The figure shows three views and two pictorial views of one solid part (mm, origin at its lowest corner). Answer the questions. Coordinates: 2 decimals unless noted, no trailing zeros. Order: outer loops, then holes, each group sorted by start corner. A loop starts at its lowest first (then second) coordinate and runs counter-clockwise, first axis right, second up. Notation, with made-up numbers: M 81,6 L 131,6 A10 cw 131,10 Z; hole C 68.5,2 d10. An arc over 180 degrees is marked long. Use a Markdown table: item, result.
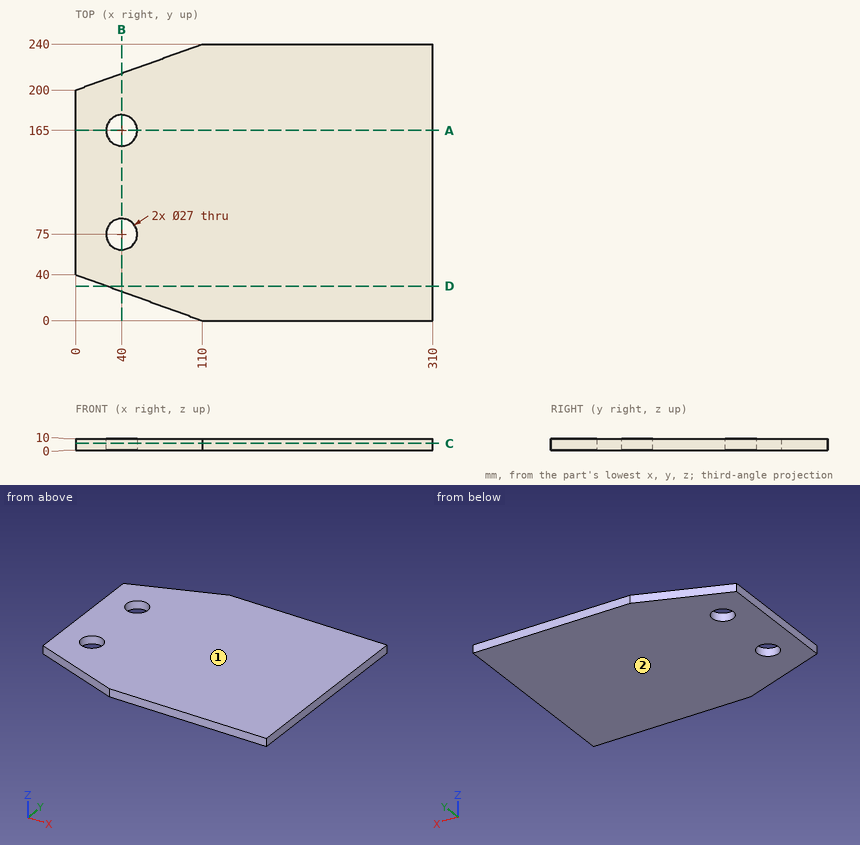
1. For a pull along Z with two mould halves and no side action, classify the marked faces 1 and 2 as +Z half, -Z half, draft (parallel to the pull), parting line (faces both ways), or undercut.
Answers below:
| item | result |
|---|---|
| face 1 | +Z half |
| face 2 | -Z half |
2. Section A-A on y = 165 is taken. Determine the outline of the cut face in (x, z), then the cut area to 3 significant figures.
Answers below:
| item | result |
|---|---|
| outline | M 0,0 L 26.5,0 L 26.5,10 L 0,10 Z; M 53.5,0 L 310,0 L 310,10 L 53.5,10 Z |
| area | 2,830 mm² |
3. Find the intervals of material crossed by probe 1 along Y at (x, z) = (40, 5.5); probe 2 along X at (y, z) = (164.5, 4.5); probe 3 along X at (y, z) = (73.5, 1.5), in increasing order.
Answers below:
| item | result |
|---|---|
| probe 1 | 25.45 to 61.5, 88.5 to 151.5, 178.5 to 214.55 |
| probe 2 | 0 to 26.51, 53.49 to 310 |
| probe 3 | 0 to 26.58, 53.42 to 310 |
4. Section C-C on z = 6 is taken. Determine the outline of the cut face in (x, y).
Answers below:
| item | result |
|---|---|
| outline | M 0,40 L 110,0 L 310,0 L 310,240 L 110,240 L 0,200 Z; hole C 40,75 d27; hole C 40,165 d27 |
5. A flat-ended cylindrical pin translates along its axis: P1, Ø21.5, axis at x = 40, y = 165, coming from the +Z side. Find the tip coordinate at first contact, or state that the pin passes through.
Answers below:
| item | result |
|---|---|
| P1 | through |
6. Section D-D on y = 30 is taken. Determine the outline of the cut face in (x, z).
Answers below:
| item | result |
|---|---|
| outline | M 27.5,0 L 310,0 L 310,10 L 27.5,10 Z |
7. Section B-B on x = 40 is taken. Determine the outline of the cut face in (y, z), then the cut area to 3 significant figures.
Answers below:
| item | result |
|---|---|
| outline | M 25.45,0 L 61.5,0 L 61.5,10 L 25.45,10 Z; M 88.5,0 L 151.5,0 L 151.5,10 L 88.5,10 Z; M 178.5,0 L 214.55,0 L 214.55,10 L 178.5,10 Z |
| area | 1,350 mm² |
